from build123d import *

# Parameters (mm, degrees)
SKETCH1_W                                           = 35.5
SKETCH1_H                                           = 30
BOSS_EXTRUDE1_DEPTH                                 = 5.25
SKETCH2_W                                           = 1.5
SKETCH2_H                                           = 27
CUT_EXTRUDE1_DEPTH                                  = 39.89489041
M5_TAPPED_HOLE1_D                                   = 4.2
M5_TAPPED_HOLE1_DEPTH                               = 12.4
M5_TAPPED_HOLE1_TIP                                 = 1.2618073
SKETCH14_OUTSIDE_W                                  = 47.03
SKETCH14_OUTSIDE_H                                  = 41.53
SKETCH14_OUTSIDE_W_2                                = 10
SKETCH14_OUTSIDE_H_2                                = 10
CUT_EXTRUDE4_DEPTH                                  = 3
CHAMFER1_SIZE                                       = 2
M4_TAPPED_HOLE3_D                                   = 3.3
M4_TAPPED_HOLE3_DEPTH                               = 10.1
M4_TAPPED_HOLE3_TIP                                 = 0.991420021
CHAMFER2_SIZE                                       = 1
CHAMFER3_SIZE                                       = 0.5
CBORE_FOR_M3_HEX_SOCKET_HEAD_CAP_SCREW1_D           = 3.4
CBORE_FOR_M3_HEX_SOCKET_HEAD_CAP_SCREW1_CBORE_D     = 6.5
CBORE_FOR_M3_HEX_SOCKET_HEAD_CAP_SCREW1_CBORE_DEPTH = 3.4
M3_TAPPED_HOLE1_D                                   = 2.5
M3_TAPPED_HOLE1_DEPTH                               = 7.5
M3_TAPPED_HOLE1_TIP                                 = 0.751075774


with BuildPart() as part:
    # Sketch1 → Boss-Extrude1 (new, symmetric)
    with BuildSketch(Plane.XY):
        Rectangle(SKETCH1_W, SKETCH1_H)
    extrude(amount=BOSS_EXTRUDE1_DEPTH, both=True)

    # Sketch2 → Cut-Extrude1 (cut, through all)
    with BuildSketch(Plane(origin=(17.75, 0, 0), x_dir=(0, 0, -1), z_dir=(1, 0, 0))):
        with Locations((-4.5, 0)):
            Rectangle(SKETCH2_W, SKETCH2_H)
    extrude(amount=-CUT_EXTRUDE1_DEPTH, mode=Mode.SUBTRACT)

    # M5 Tapped Hole1
    with Locations(Plane(origin=(0, 0, -5.25), x_dir=(-1, 0, 0), z_dir=(0, 0, -1))):
        with Locations((0, 0)):
            Hole(M5_TAPPED_HOLE1_D / 2, depth=M5_TAPPED_HOLE1_DEPTH)
            with Locations((0, 0, -(M5_TAPPED_HOLE1_DEPTH + M5_TAPPED_HOLE1_TIP / 2))):  # 118° drill point
                Cone(0, M5_TAPPED_HOLE1_D / 2, M5_TAPPED_HOLE1_TIP, mode=Mode.SUBTRACT)

    # Sketch14 outside → Cut-Extrude4 (cut)
    with BuildSketch(Plane(origin=(0, 0, -5.25), x_dir=(-1, 0, 0), z_dir=(0, 0, -1))):
        Rectangle(SKETCH14_OUTSIDE_W, SKETCH14_OUTSIDE_H)
        Rectangle(SKETCH14_OUTSIDE_W_2, SKETCH14_OUTSIDE_H_2, mode=Mode.SUBTRACT)
    extrude(amount=-CUT_EXTRUDE4_DEPTH, mode=Mode.SUBTRACT)

    # Chamfer1
    chamfer1_edges = [part.edges().sort_by_distance(p)[0] for p in [
        (5, 5, -3.75),
        (-5, 5, -3.75),
        (-5, -5, -3.75),
        (5, -5, -3.75),
    ]]
    chamfer(chamfer1_edges, length=CHAMFER1_SIZE)

    # M4 Tapped Hole3
    with Locations(Plane(origin=(0, 0, -2.25), x_dir=(-1, 0, 0), z_dir=(0, 0, -1))):
        with Locations((-12.75, 4), (-12.75, -4)):
            Hole(M4_TAPPED_HOLE3_D / 2, depth=M4_TAPPED_HOLE3_DEPTH)
            with Locations((0, 0, -(M4_TAPPED_HOLE3_DEPTH + M4_TAPPED_HOLE3_TIP / 2))):  # 118° drill point
                Cone(0, M4_TAPPED_HOLE3_D / 2, M4_TAPPED_HOLE3_TIP, mode=Mode.SUBTRACT)

    # Chamfer2
    chamfer2_edges = [part.edges().sort_by_distance(p)[0] for p in [
        (17.75, -15, 1.5),
        (-17.75, -15, 1.5),
        (-17.75, 15, 1.5),
        (17.75, 15, 1.5),
    ]]
    chamfer(chamfer2_edges, length=CHAMFER2_SIZE)

    # Chamfer3
    chamfer3_edges = [part.edges().sort_by_distance(p)[0] for p in [
        (-2.1, 0, -5.25),
        (5, 0, -5.25),
        (0, 5, -5.25),
        (0, -5, -5.25),
        (-5, 0, -5.25),
        (-4, -4, -5.25),
        (-4, 4, -5.25),
        (4, 4, -5.25),
        (4, -4, -5.25),
    ]]
    chamfer(chamfer3_edges, length=CHAMFER3_SIZE)

    # CBORE for M3 Hex Socket Head Cap Screw1 (through all)
    with Locations(Plane(origin=(0, 0, -2.25), x_dir=(-1, 0, 0), z_dir=(0, 0, -1))):
        with Locations((-7.5, 10), (7.5, 10), (7.5, -10), (-7.5, -10)):
            CounterBoreHole(CBORE_FOR_M3_HEX_SOCKET_HEAD_CAP_SCREW1_D / 2, CBORE_FOR_M3_HEX_SOCKET_HEAD_CAP_SCREW1_CBORE_D / 2, CBORE_FOR_M3_HEX_SOCKET_HEAD_CAP_SCREW1_CBORE_DEPTH)

    # M3 Tapped Hole1
    with Locations(Plane(origin=(-17.75, -2.75, 0), x_dir=(0, -1, 0), z_dir=(-1, 0, 0))):
        with Locations((3.25, 1.5), (-8.75, 1.5)):
            Hole(M3_TAPPED_HOLE1_D / 2, depth=M3_TAPPED_HOLE1_DEPTH)
            with Locations((0, 0, -(M3_TAPPED_HOLE1_DEPTH + M3_TAPPED_HOLE1_TIP / 2))):  # 118° drill point
                Cone(0, M3_TAPPED_HOLE1_D / 2, M3_TAPPED_HOLE1_TIP, mode=Mode.SUBTRACT)


solid = part.part
The model under review builds one solid part; all positions refer to its coordinate system, in mm. A direction names the side the tool comes from. Round coordinates to 2 decimals unless told otherwise and drop trailing zeros. Write each loop counter-clockwise with the first axis right and the second up, starting at its lowest first coordinate (ties: lowest second). Pieces come first, ordered by that corner, then holes. Notation, with made-up numbers: (-5, -23.75) -> (34, -23.75) arc R25 ccw to (34, -2.75) -> close; hole circle Ø3 at (84.25, 18.5). An arc over 180 degrees is marked (long way). Answer as a JSON object with one key per item and string values.
1. We need section C-C on x = 12.75. State the section outline as (y, z) points.
Results found:
{"outline": "(-15, -2.25) -> (-5.65, -2.25) -> (-5.65, 3.75) -> (-13.5, 3.75) -> (-13.5, 5.25) -> (-15, 5.25) -> close; (-2.35, -2.25) -> (2.35, -2.25) -> (2.35, 3.75) -> (-2.35, 3.75) -> close; (5.65, -2.25) -> (15, -2.25) -> (15, 5.25) -> (13.5, 5.25) -> (13.5, 3.75) -> (5.65, 3.75) -> close"}
2. To check wall thickness, follow line 1 along Y through (x, z) = (12.75, 1); line 2 along Y through (x, z) = (7.5, -1.5); line 3 along Z through (x, y) = (-12.5, -6). State the ranges of each line that lie inside material, in increasing order.
Results found:
{"line 1": "y = -15 to -5.65, -2.35 to 2.35, 5.65 to 15", "line 2": "y = -15 to -13.25, -6.75 to 6.75, 13.25 to 15", "line 3": "z = -2.25 to 0.25, 2.75 to 3.75"}
3. The part is to be moulded in two halves that separate along X. For faces 1 (the face through (-5.105, -7.803, -0.574)), 2 (the face through (6.1, 8.6, 1.15)), 3 (the face through (3.835, 3.807, -5.004)), 4 (the face through (0, -5, -4)), say which applies: pulls with the +X half, pulls with the -X half, needs draft (parallel to the pull), parting line crosses it, or undercut.
Results found:
{"face 1": "undercut", "face 2": "undercut", "face 3": "pulls with the +X half", "face 4": "needs draft"}
4. We need section B-B on x = -15.5. State the section outline as (y, z) points.
Results found:
{"outline": "(-15, -2.25) -> (15, -2.25) -> (15, 5.25) -> (13.5, 5.25) -> (13.5, 3.75) -> (-13.5, 3.75) -> (-13.5, 5.25) -> (-15, 5.25) -> close; hole circle Ø2.5 at (-6, 1.5); hole circle Ø2.5 at (6, 1.5)"}
5. We need section A-A on y = 10. State the section outline as (x, z) points.
Results found:
{"outline": "(-17.75, -2.25) -> (-10.75, -2.25) -> (-10.75, 1.15) -> (-9.2, 1.15) -> (-9.2, 3.75) -> (-17.75, 3.75) -> close; (-5.8, 1.15) -> (-4.25, 1.15) -> (-4.25, -2.25) -> (4.25, -2.25) -> (4.25, 1.15) -> (5.8, 1.15) -> (5.8, 3.75) -> (-5.8, 3.75) -> close; (9.2, 1.15) -> (10.75, 1.15) -> (10.75, -2.25) -> (17.75, -2.25) -> (17.75, 3.75) -> (9.2, 3.75) -> close"}
6. We need section D-D on z = -4. State the section outline as (x, y) points.
Results found:
{"outline": "(-5, -3) -> (-3, -5) -> (3, -5) -> (5, -3) -> (5, 3) -> (3, 5) -> (-3, 5) -> (-5, 3) -> close; hole circle Ø4.2 at (0, 0)"}
7. Machinability: for faces 5 (the face through (4, -4, -4)), 6 (the face through (0, 3, 3.75)), 7 (the face through (6.1, -11.4, 1.15)), which of the approach directions +Z, -Z, +X, -X, +Y, -Y give a long, thin tool a straight path to every point of the face, cutting with its end or side? Answer none if there is none.
Results found:
{"face 5": "-Z, +X, -Y", "face 6": "+Z, +X, -X", "face 7": "-Z"}
8. Clearance check with flat-ended pins moving along their axes: pin 1 (5.5 mm diameter, centred on x = 0, y = 0, fed in from +Z); pin 2 (5 mm diameter, centred on x = 8, y = -11, fed in from -Z); pin 3 (4.5 mm diameter, centred on x = -7.5, y = -10, fed in from -Z). State where each tip first meets the part, or that it passes through.
Results found:
{"pin 1": "stops at z = 3.75", "pin 2": "stops at z = -2.25", "pin 3": "stops at z = 1.15"}
